from build123d import *

# Parameters (mm, degrees)
SKETCH4_R           = 2.5
BOSS_EXTRUDE3_DEPTH = 4
FILLET2_R           = 5
SKETCH7_R           = 3.986171954
SKETCH7_R_2         = 1.5
BOSS_EXTRUDE4_DEPTH = 4
BOSS_EXTRUDE5_DEPTH = 4
SKETCH9_R           = 1.5
CUT_EXTRUDE1_DEPTH  = 27.524941093
BOSS_EXTRUDE6_DEPTH = 4


with BuildPart() as part:
    # Sketch4 → Boss-Extrude3 (new body)
    with BuildSketch(Plane.XY):
        with BuildLine():
            Line((0, -20.5), (0, -4.15))
            ThreePointArc((0, -4.15), (8.175, 4.025), (0, 12.2))
            ThreePointArc((0, 12.2), (-16.35, -4.15), (0, -20.5))
        make_face()
        Circle(SKETCH4_R, mode=Mode.SUBTRACT)
    extrude(amount=BOSS_EXTRUDE3_DEPTH)

    # Fillet2
    fillet2_edges = [part.edges().sort_by_distance(p)[0] for p in [
        (0, -4.15, 2),
    ]]
    fillet(fillet2_edges, radius=FILLET2_R)

    # Sketch7 → Boss-Extrude4 (add)
    with BuildSketch(Plane.XY.offset(4)):
        Circle(SKETCH7_R)
        Circle(SKETCH7_R_2, mode=Mode.SUBTRACT)
    extrude(amount=-BOSS_EXTRUDE4_DEPTH)

    # Sketch8 → Boss-Extrude5 (add)
    with BuildSketch(Plane.XY.offset(4)):
        Polygon((0, 0), (-1, 1.118033989), (-1.075164003, 1.990831029), (0.996128458, 2.028687549), (1.118033989, 1), align=None)
    extrude(amount=-BOSS_EXTRUDE5_DEPTH)

    # Sketch9 → Cut-Extrude1 (cut, through all)
    with BuildSketch(Plane.XY.offset(4)):
        Circle(SKETCH9_R)
    extrude(amount=-CUT_EXTRUDE1_DEPTH, mode=Mode.SUBTRACT)

    # Sketch10 → Boss-Extrude6 (add, through all)
    with BuildSketch(Plane.XY.offset(4)):
        with BuildLine():
            ThreePointArc((1.5, 0), (1.299038106, 0.75), (0.75, 1.299038106))
            Line((0.75, 1.299038106), (0.75, -1.299038106))
            ThreePointArc((0.75, -1.299038106), (1.299038106, -0.75), (1.5, 0))
        make_face()
        with BuildLine():
            Line((-0.75, -1.299038106), (-0.75, 1.299038106))
            ThreePointArc((-0.75, 1.299038106), (-1.5, 0), (-0.75, -1.299038106))
        make_face()
    extrude(amount=-BOSS_EXTRUDE6_DEPTH)


solid = part.part
Could you check a few things on this model? Use its own coordinates, in mm. A direction names the side the tool comes from. Give positions to 0.01 mm unless a question says otherwise; leave off trailing zeros. Order: outer loops, then holes, each group sorted by start corner. A loop starts at its lowest first (then second) coordinate and runs counter-clockwise, first axis right, second up. Notation, with made-up numbers: (27, -21) -> (40, -21) arc R25 cw to (40, 4) -> close; hole circle Ø7 at (38, 73.5). An arc over 180 degrees is marked (long way). Return JSON: item names as keys, results as strings.
1. Imagine slicing it at C-C on y = -7. List the corners of the cut face in (x, z) for me.
Answer list:
{"outline": "(-16.1, 0) -> (0.14, 0) -> (0.14, 4) -> (-16.1, 4) -> close"}
2. Imagine slicing it at A-A on z = 0.5. List the corners of the cut face in (x, y) for me (3 decimals).
Answer list:
{"outline": "(0, -20.5) -> (0, -8.164) arc R5 cw to (3.102, -3.538) arc R8.175 ccw to (0, 12.2) arc R16.35 ccw to start; hole (-0.75, -1.299) arc R1.5 ccw to (0.75, -1.299) -> (0.75, 1.299) arc R1.5 ccw to (-0.75, 1.299) -> close"}
3. Imagine slicing it at B-B on y = 3. List the corners of the cut face in (x, z) for me, then the cut area to 3 significant figures.
Answer list:
{"outline": "(-14.7, 0) -> (8.11, 0) -> (8.11, 4) -> (-14.7, 4) -> close", "area": "91.3 mm2"}
4. For pin 1 Ø2 at (y, z) = (0, 2) entering from +X; pin 2 Ø0.8 at (y, z) = (-0.5, 1.5) entering from -X; pin 3 Ø2 at (x, z) = (-12.5, 3) entering from +Y, each with a flat end and sliding along its axis, tell me the tip position at first contact or that it passes through.
Answer list:
{"pin 1": "stops at x = 7.59", "pin 2": "stops at x = -16.02", "pin 3": "stops at y = 7.47"}
5. On a 3-axis mill with a long thin cutter (end or side, diameter ignored), from which of +Z, -Z, +X, -X, +Y, -Y can I reach the whole of each face in a straight line? I mean faces 1 (the cylindrical face through (0, -1.5, 2)), 2 (the cylindrical face through (8.05, 5.45, 1.97)). Say none if no direction works.
Answer list:
{"face 1": "+Z, -Z", "face 2": "+Z, -Z, +X"}
6. Thinking about a two-plate mould opening in X: for faces 3 (the flat face through (0.75, 0, 2)), 4 (the flat face through (-4, -4, 4)), 5 (the cylindrical face through (0, 1.5, 2)), 6 (the flat face through (0, -14, 2)), which applies, pulls with the +X half, pulls with the -X half, needs draft (parallel to the pull), parting line crosses it, or undercut?
Answer list:
{"face 3": "undercut", "face 4": "needs draft", "face 5": "undercut", "face 6": "pulls with the +X half"}
7. I need wall thicknesses on line 1 (X direction, y = 0, z = 0.85); line 2 (X direction, y = -6, z = 0.2) (3 decimals); line 3 (Y direction, x = -13.75, z = 1.8). Which ranges of each line are inside material? Lowest first, please. Write a range as from..to.
Answer list:
{"line 1": "x = -15.81..-0.75, 0.75..7.12", "line 2": "x = -16.245..0.493", "line 3": "y = -13..4.7"}
